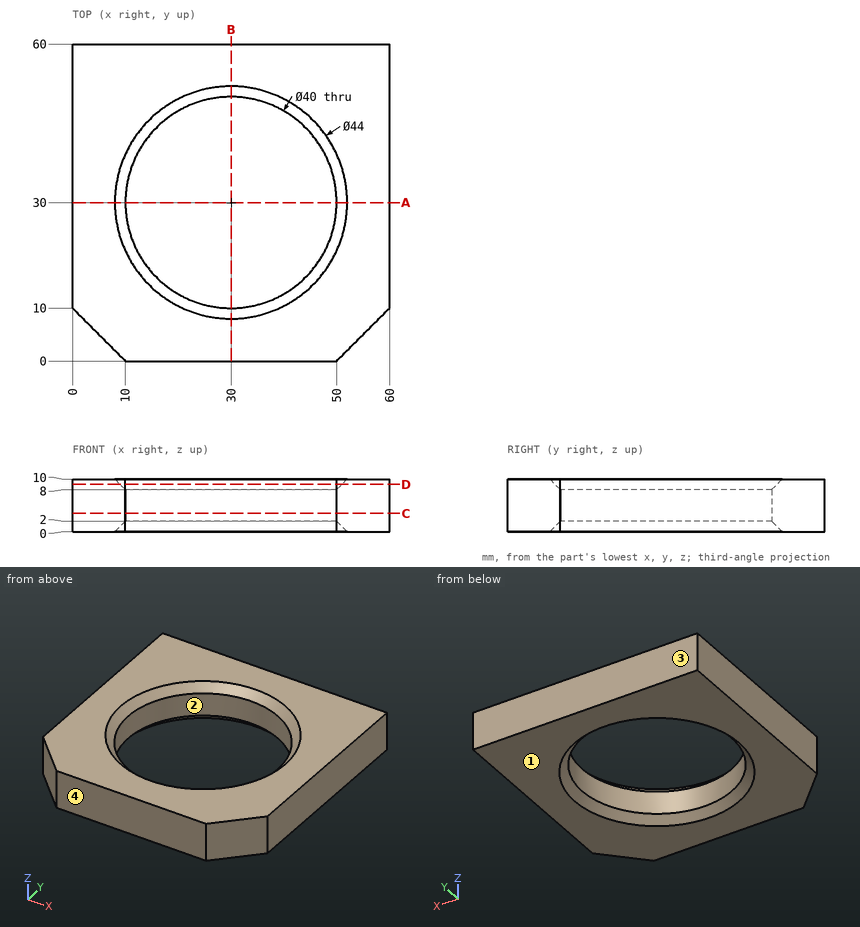
Part print with two shaded views. Sizes in mm from the minimum x, y, z corner. Coordinates: 2 decimals unless noted, no trailing zeros. Write each loop counter-clockwise with the first axis right and the second up, starting at its lowest first coordinate (ties: lowest second). Pieces come first, ordered by that corner, then holes. Notation, with made-up numbers: (53.5, 47.25) - (71.5, 47.25) arc R20 cw to (71.5, 68.25) - close; hole circle Ø10 at (87, -31.5). An arc over 180 degrees is marked (long way). Use a Markdown table: item, result. Add a question column.
Item 1: Drill centre lines: line 1 along X through (y, z) = (15.5, 9.25); line 2 along X through (y, z) = (12.5, 2.25); line 3 along Y through (x, z) = (45, 6.75). Where is each one in solid material? Low to high.
Item 2: Two-plate mould, pull along Y, no slides. Class the marked faces 1, 2, 3 and 4: pulls with the +Y half, pulls with the -Y half, needs draft (parallel to the pull), parting line crosses it, or undercut.
Item 3: Band-saw the part on D-D, the plane z = 9. Write the cut outline in (x, y).
Item 4: Band-saw the part on C-C, the plane z = 3.5. Write the cut outline in (x, y).
Item 5: Band-saw the part on A-A, the plane y = 30. Write the cut outline in (x, z), and give its area (3 significant figures).
A:
| question | item | result |
|---|---|---|
| 1 | line 1 | x = 0 to 14.47, 45.53 to 60 |
| 1 | line 2 | x = 0 to 20.32, 39.68 to 60 |
| 1 | line 3 | y = 0 to 16.77, 43.23 to 60 |
| 2 | face 1 | needs draft |
| 2 | face 2 | undercut |
| 2 | face 3 | pulls with the +Y half |
| 2 | face 4 | pulls with the -Y half |
| 3 | outline | (0, 10) - (10, 0) - (50, 0) - (60, 10) - (60, 60) - (0, 60) - close; hole circle Ø42 at (30, 30) |
| 4 | outline | (0, 10) - (10, 0) - (50, 0) - (60, 10) - (60, 60) - (0, 60) - close; hole circle Ø40 at (30, 30) |
| 5 | outline | (0, 0) - (8, 0) - (10, 2) - (10, 8) - (8, 10) - (0, 10) - close; (50, 2) - (52, 0) - (60, 0) - (60, 10) - (52, 10) - (50, 8) - close |
| 5 | area | 192 mm² |
